from build123d import *

# Parameters (mm, degrees)
EXTRUDE_1_DEPTH      = 30
EXTRUDE_1_DEPTH_BACK = 15
SKETCH_1_R           = 7.5
SKETCH_2_R           = 7.5
SKETCH_2_R_2         = 3
CUT_EXTRUDE_1_DEPTH  = 10
CHAMFER_1_SIZE       = 1
SKETCH_3_R           = 7.5
SKETCH_3_R_2         = 6
CUT_EXTRUDE_2_DEPTH  = 15
CHAMFER_2_SIZE       = 1
CHAMFER_3_SIZE       = 1
CHAMFER_4_SIZE       = 1
SKETCH_4_W           = 26.213765936
SKETCH_4_H           = 7.269713565
SKETCH_4_W_2         = 30.615700216
SKETCH_4_H_2         = 9.339731857
CUT_EXTRUDE_3_DEPTH  = 5


with BuildPart() as part:
    # 草图1 → 凸台-拉伸1 (new, two sides: drawn at the far end of the back side and taken through both)
    with BuildSketch(Plane.XY.offset(-EXTRUDE_1_DEPTH_BACK)):
        Circle(SKETCH_1_R)
    extrude(amount=EXTRUDE_1_DEPTH + EXTRUDE_1_DEPTH_BACK)

    # 草图2 → 切除-拉伸1 (cut)
    with BuildSketch(Plane.XY.offset(30)):
        Circle(SKETCH_2_R)
        Circle(SKETCH_2_R_2, mode=Mode.SUBTRACT)
    extrude(amount=-CUT_EXTRUDE_1_DEPTH, mode=Mode.SUBTRACT)

    # 倒角1
    chamfer_1_edges = [part.edges().sort_by_distance(p)[0] for p in [
        (-3, 0, 30),
    ]]
    chamfer(chamfer_1_edges, length=CHAMFER_1_SIZE)

    # 草图3 → 切除-拉伸2 (cut)
    with BuildSketch(Plane(origin=(0, 0, -15), x_dir=(-1, 0, 0), z_dir=(0, 0, -1))):
        with Locations(Location((0, 0, 0), (0, 0, 180))):
            Circle(SKETCH_3_R)
        Circle(SKETCH_3_R_2, mode=Mode.SUBTRACT)
    extrude(amount=-CUT_EXTRUDE_2_DEPTH, mode=Mode.SUBTRACT)

    # 倒角2
    chamfer_2_edges = [part.edges().sort_by_distance(p)[0] for p in [
        (6, 0, -15),
    ]]
    chamfer(chamfer_2_edges, length=CHAMFER_2_SIZE)

    # 倒角3
    chamfer_3_edges = [part.edges().sort_by_distance(p)[0] for p in [
        (-7.5, 0, 0),
    ]]
    chamfer(chamfer_3_edges, length=CHAMFER_3_SIZE)

    # 倒角4
    chamfer_4_edges = [part.edges().sort_by_distance(p)[0] for p in [
        (-7.5, 0, 20),
    ]]
    chamfer(chamfer_4_edges, length=CHAMFER_4_SIZE)

    # 草图4 → 切除-拉伸3 (cut)
    with BuildSketch(Plane.XY.offset(20)):
        with Locations((-1.405852491, -8.634856782)):
            Rectangle(SKETCH_4_W, SKETCH_4_H)
        with Locations((-0.14462413, 9.669865929)):
            Rectangle(SKETCH_4_W_2, SKETCH_4_H_2)
    extrude(amount=-CUT_EXTRUDE_3_DEPTH, mode=Mode.SUBTRACT)


solid = part.part
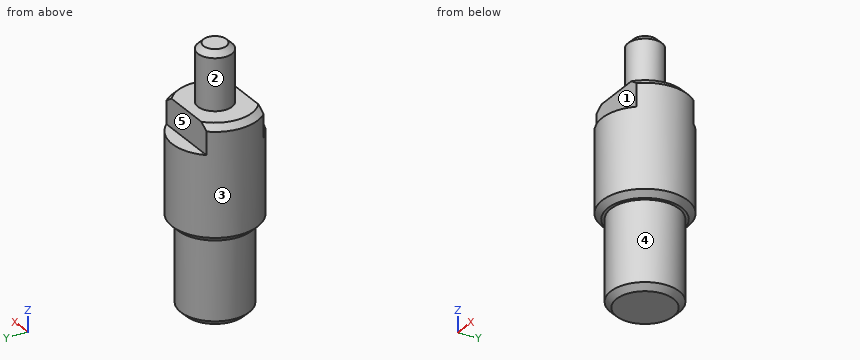
Source: CAD feature listing. Evaluate the final solid. Frame: model axes, mm. Face numbers are marked on the shaded views. A direction names the side the tool comes from. Coordinates: 2 decimals unless noted, no trailing zeros. Loops run counter-clockwise (first coordinate to the right, second up) from the corner with the lowest first, then second, coordinate; pieces in that order, holes last. Notation, with made-up numbers: M 85,3.5 L 125,3.5 A35 ccw 125,38.5 Z; hole C 41,46.25 d6. An arc over 180 degrees is marked long. Answer in a Markdown table with one row per item.
Q1. Set-up query: the marked faces 1, 2, 3, 4 and 5. Return all of +Z, -Z, +X, -X, +Y, -Y with unobstructed straight access to the full face (end or side cutting, diameter ignored); none if empty.
Answers below:
| item | result |
|---|---|
| face 1 | +Z, +X, -X, -Y |
| face 2 | +Z |
| face 3 | +Z, -Z |
| face 4 | -Z |
| face 5 | +Z, +X, -X, +Y |
Q2. Section C-C on z = 24. Return the cut outline in (x, y).
Answers below:
| item | result |
|---|---|
| outline | C 0,0 d6 |
Q3. Ray query, probe 1 along X at (y, z) = (5, 14); probe 2 along Z at (x, y) = (-1, 4); probe 3 along Y at (x, z) = (0.5, 17). Return the intervals inside material, ascending. Write a range as from..to.
Answers below:
| item | result |
|---|---|
| probe 1 | x = -5.59..5.59 |
| probe 2 | z = -15..20 |
| probe 3 | y = -5..5 |
Q4. Section B-B on x = 0. Return the cut outline in (y, z), plus the area to 3 significant figures.
Answers below:
| item | result |
|---|---|
| outline | M -7.5,1 L -6.5,0 L -6,0 L -6,-14 L -5,-15 L 5,-15 L 6,-14 L 6,0 L 6.5,0 L 7.5,1 L 7.5,15 L 5,15 L 5,20 L 3,20 L 3,29 L 2,30 L -2,30 L -3,29 L -3,20 L -5,20 L -5,15 L -7.5,15 Z |
| area | 512 mm^2 |
Q5. Section D-D on z = 6. Return the cut outline in (x, y), plus the area to 3 significant figures.
Answers below:
| item | result |
|---|---|
| outline | C 0,0 d15 |
| area | 177 mm^2 |
Q6. First-contact query: pin 1 (0.7 mm diameter, centred on x = 0, y = 6, fed in from +Z); pin 2 (2 mm diameter, centred on y = 2.5, z = 15, fed in from -X); pin 3 (4 mm diameter, centred on x = 4, z = 22.5, fed in from -Y). Flat tips, straight axial feed; report the tip coordinate or a pass-through.
Answers below:
| item | result |
|---|---|
| pin 1 | stops at z = 15 |
| pin 2 | stops at x = -7.35 |
| pin 3 | stops at y = -2.24 |
Q7. Section A-A on y = 0. Return the cut outline in (x, z).
Answers below:
| item | result |
|---|---|
| outline | M -7.5,1 L -6.5,0 L -6,0 L -6,-14 L -5,-15 L 5,-15 L 6,-14 L 6,0 L 6.5,0 L 7.5,1 L 7.5,19 L 6.5,20 L 3,20 L 3,29 L 2,30 L -2,30 L -3,29 L -3,20 L -6.5,20 L -7.5,19 Z |
